Verification items for the finished model (mm, model axes). A direction names the side the tool comes from. Coordinates: 2 decimals unless noted, no trailing zeros. Order: outer loops, then holes, each group sorted by start corner. A loop starts at its lowest first (then second) coordinate and runs counter-clockwise, first axis right, second up. Notation, with made-up numbers: M -7,-13.75 L 42,-13.75 A16 cw 42,5.25 Z; hole C 85.25,76 d3. An arc over 180 degrees is marked long. Return JSON: item names as keys, results as strings. Group by question number.
1. Material ranges on line 1 along Y through (x, z) = (2, 1163.5); line 2 along Y through (x, z) = (17, 540); line 3 along X through (y, z) = (2, 382), recorded low to high.
2. Set-up check for faces 1 (the flat face through (-11.3, 22.4, 1120)), 2 (the flat face through (0, 0, 1240)), 3 (the flat face through (-11.3, 22.4, 120)): record each of +Z, -Z, +X, -X, +Y, -Y from which the full face is reachable in a straight line by a thin tool's end or side.
3. Gauge pin test, flat ends, axial feed: pin 1 (5 mm diameter, centred on y = -16, z = 804, fed in from +X); pin 2 (8 mm diameter, centred on y = -17.5, z = 337, fed in from -X); pin 3 (1.5 mm diameter, centred on x = 2.5, z = 908.5, fed in from -Y). Record the tip position at first contact, or that the pin passes through.
4. Section check C-C, the plane z = 995.5. Record the cut outline in (x, y).
5. Section check A-A, the plane x = 0. Record the cut outline in (y, z), plus the area to 3 significant figures.
```python
from build123d import *

# Parameters (mm, degrees)
SKETCH1_R           = 21
BOSS_EXTRUDE1_DEPTH = 85
SKETCH2_R           = 24.8
BOSS_EXTRUDE2_DEPTH = 35
SKETCH3_R           = 30
BOSS_EXTRUDE3_DEPTH = 1000
SKETCH4_R           = 24.8
BOSS_EXTRUDE4_DEPTH = 30
SKETCH5_R           = 21
BOSS_EXTRUDE5_DEPTH = 90
CHAMFER2_SIZE       = 2


with BuildPart() as part:
    # Sketch1 → Boss-Extrude1 (new body)
    with BuildSketch(Plane.XY):
        Circle(SKETCH1_R)
    extrude(amount=BOSS_EXTRUDE1_DEPTH)

    # Sketch2 → Boss-Extrude2 (add)
    with BuildSketch(Plane.XY.offset(85)):
        Circle(SKETCH2_R)
    extrude(amount=BOSS_EXTRUDE2_DEPTH)

    # Sketch3 → Boss-Extrude3 (add)
    with BuildSketch(Plane.XY.offset(120)):
        Circle(SKETCH3_R)
    extrude(amount=BOSS_EXTRUDE3_DEPTH)

    # Sketch4 → Boss-Extrude4 (add)
    with BuildSketch(Plane.XY.offset(1120)):
        Circle(SKETCH4_R)
    extrude(amount=BOSS_EXTRUDE4_DEPTH)

    # Sketch5 → Boss-Extrude5 (add)
    with BuildSketch(Plane.XY.offset(1150)):
        Circle(SKETCH5_R)
    extrude(amount=BOSS_EXTRUDE5_DEPTH)

    # Chamfer2
    chamfer2_edges = [part.edges().sort_by_distance(p)[0] for p in [
        (-24.8, 0, 1150),
        (-21, 0, 1240),
        (-21, 0, 0),
        (-24.8, 0, 85),
    ]]
    chamfer(chamfer2_edges, length=CHAMFER2_SIZE)


solid = part.part
```
Answers follow:
{
 "1": {"line 1": "-20.9 to 20.9", "line 2": "-24.72 to 24.72", "line 3": "-29.93 to 29.93"},
 "2": {"face 1": "+Z", "face 2": "+Z, +X, -X, +Y, -Y", "face 3": "-Z"},
 "3": {"pin 1": "x = 26.79", "pin 2": "x = -26.79", "pin 3": "y = -29.95"},
 "4": {"outline": "C 0,0 d60"},
 "5": {"outline": "M -30,120 L -24.8,120 L -24.8,87 L -22.8,85 L -21,85 L -21,2 L -19,0 L 19,0 L 21,2 L 21,85 L 22.8,85 L 24.8,87 L 24.8,120 L 30,120 L 30,1120 L 24.8,1120 L 24.8,1148 L 22.8,1150 L 21,1150 L 21,1238 L 19,1240 L -19,1240 L -21,1238 L -21,1150 L -22.8,1150 L -24.8,1148 L -24.8,1120 L -30,1120 Z", "area": "70,600 mm^2"}
}
